Could you check a few things on this drawing? It's one solid part, dimensions in mm from its lowest x, y, z. A direction names the side the tool comes from. Give positions to 0.01 mm unless a question says otherwise; leave off trailing zeros. Order: outer loops, then holes, each group sorted by start corner. A loop starts at its lowest first (then second) coordinate and runs counter-clockwise, first axis right, second up. Notation, with made-up numbers: M -39,-15.5 L 16,-15.5 A20 cw 16,20.5 Z; hole C 45,5.25 d9. An arc over 180 degrees is marked long. One line per item, written item: value. Start each with the question number.
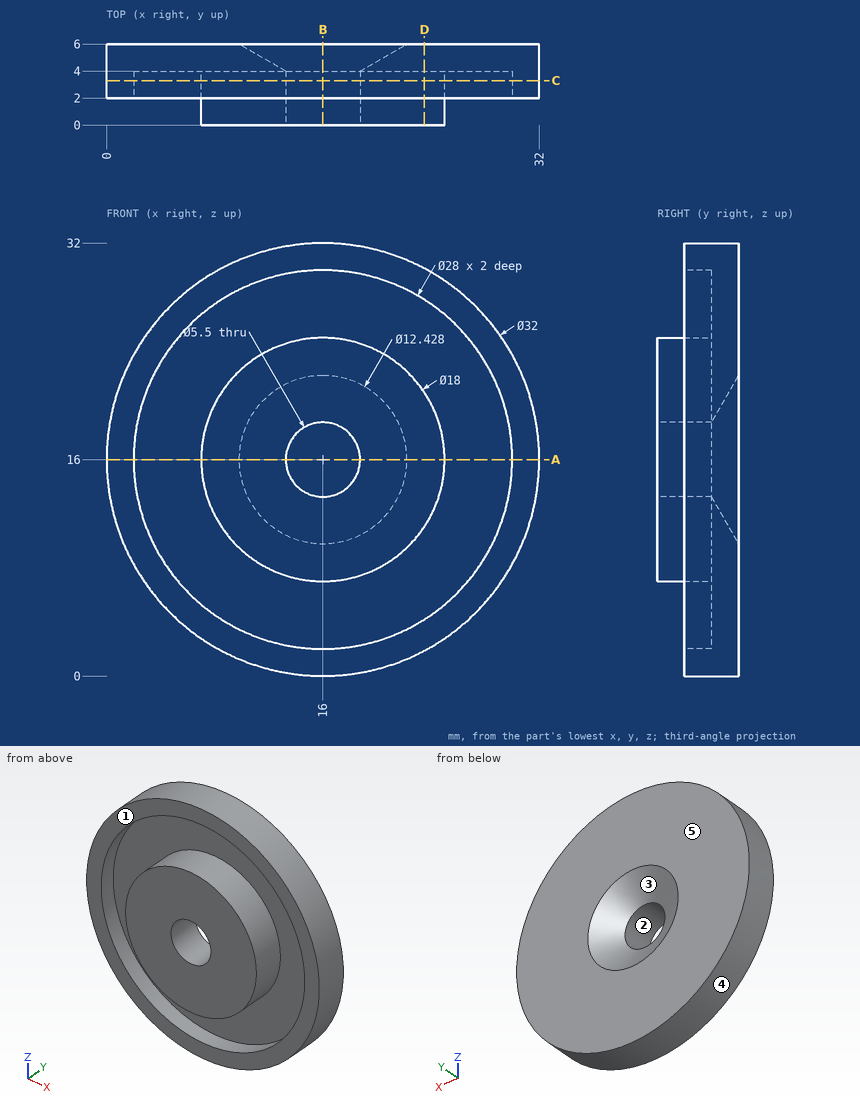
Item 1: I want a section at D-D on x = 23.5. Write out the boundary of the cut face in (y, z) (1 decimal), plus the area to 3 significant figures.
Item 2: Will these pins go through, and if not, where does the flat tip stop? P1, Ø4, axis at x = 3.5, z = 17.5, coming from the -Y side; P2, Ø1.5, axis at x = 14, y = 2.5, coming from the +Z side; P3, Ø3.5, axis at x = 16, z = 16, coming from the -Y side; P4, Ø2, axis at y = 3, z = 26, coming from the -X side.
Item 3: Please list where these lines run through material, in increasing order: probe 1 along X at (y, z) = (2.8, 16); probe 2 along Z at (x, y) = (17, 3.95) (1 decimal); probe 3 along X at (y, z) = (0.85, 16). Write a range as [from, to].
Item 4: I want a section at C-C on y = 3.3. Write out the boundary of the cut face in (x, z).
Item 5: I want a section at B-B on x = 16. Write out the boundary of the cut face in (y, z), plus the area to 3 significant figures.
Item 6: I want a section at A-A on z = 16. Write out the boundary of the cut face in (x, y), plus the area to 3 significant figures.
Item 7: For the marked faces 1 and 2, which set-ups out of +Z, -Z, +X, -X, +Y, -Y let a thin tool reach every point of the face, with its end or its side?
Item 8: We'd pull the mould along Z, two halves only. Please class the marked faces 3, 4 and 5: +Z half, -Z half, draft (parallel to the pull), parting line (faces both ways), or undercut.
Answer below:
1. outline: M 0,11 L 4,11 L 4,4.2 L 2,4.2 L 2,1.9 L 6,1.9 L 6,30.1 L 2,30.1 L 2,27.8 L 4,27.8 L 4,21 L 0,21 Z
1. area: 106 mm²
2. P1: stops at y = 2
2. P2: stops at z = 31.95
2. P3: passes through
2. P4: stops at x = 2.77
3. probe 1: x = [0, 2], [7, 13.25], [18.75, 25], [30, 32]
3. probe 2: z = [0, 2], [7.1, 13.4], [18.6, 24.9], [30, 32]
3. probe 3: x = [7, 13.25], [18.75, 25]
4. outline: C 16,16 d32; C 16,16 d18; hole C 16,16 d28; hole C 16,16 d5.5
5. outline: M 0,7 L 4,7 L 4,2 L 2,2 L 2,0 L 6,0 L 6,9.79 L 4,13.25 L 0,13.25 Z; M 0,18.75 L 4,18.75 L 6,22.21 L 6,32 L 2,32 L 2,30 L 4,30 L 4,25 L 0,25 Z
5. area: 104 mm²
6. outline: M 0,2 L 2,2 L 2,4 L 7,4 L 7,0 L 13.25,0 L 13.25,4 L 9.79,6 L 0,6 Z; M 18.75,0 L 25,0 L 25,4 L 30,4 L 30,2 L 32,2 L 32,6 L 22.21,6 L 18.75,4 Z
6. area: 104 mm²
7. face 1: -Y
7. face 2: +Y, -Y
8. face 3: undercut
8. face 4: parting line
8. face 5: draft
